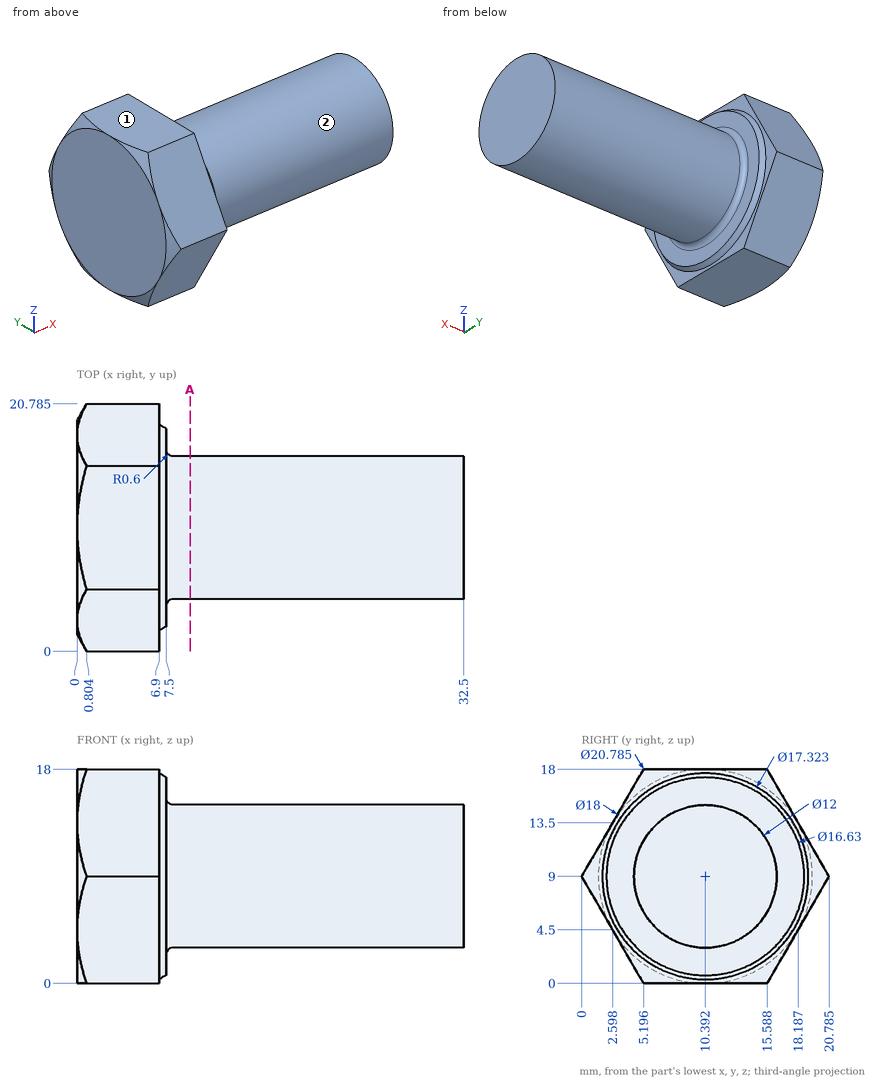
Geometry check sheet. Reference: drawing and pictorial views, mm from the part's lowest x, y, z. A direction names the side the tool comes from. Coordinates: 2 decimals unless noted, no trailing zeros. Loops run counter-clockwise (first coordinate to the right, second up) from the corner with the lowest first, then second, coordinate; pieces in that order, holes last.
1) Material ranges on probe 1 along Y at (x, z) = (28.5, 9.25); probe 2 along X at (y, z) = (6.25, 16); probe 3 along X at (y, z) = (6.5, 14), recorded low to high.
2) Access from +Z, -Z, +X, -X, +Y, -Y to the whole of each face (thin tool, end or side, straight path). Record for the marked faces 1 and 2.
3) Sectioned sample at A-A (x = 9.5). Record the boundary of the cut face in (y, z), and give its area (3 significant figures).
4) Gauge pin test, flat ends, axial feed: pin 1 (2 mm diameter, centred on x = 27, z = 7.5, fed in from +Y); pin 2 (1 mm diameter, centred on y = 16.5, z = 3, fed in from +X); pin 3 (4 mm diameter, centred on x = 11.5, y = 7.5, fed in from -Z). Record the tip position at first contact, or that the pin passes through.
Check sheet entries:
1. probe 1: y = 4.4 to 16.39
1. probe 2: x = 0 to 7.5
1. probe 3: x = 0 to 7.56
2. face 1: +Z, +X, -X, +Y, -Y
2. face 2: +X
3. outline: circle Ø12 at (10.39, 9)
3. area: 113 mm2
4. pin 1: stops at y = 16.37
4. pin 2: stops at x = 7.5
4. pin 3: stops at z = 3.07
